Input: part model. Units: mm. Frame: model coordinates. A direction names the side the tool comes from. Coordinates: 2 decimals unless noted, no trailing zeros. Order: outer loops, then holes, each group sorted by start corner. A loop starts at its lowest first (then second) coordinate and runs counter-clockwise, first axis right, second up.
from build123d import *

# Parameters (mm, degrees)
SWEEP1_PROFILE_R = 9.5
CHAMFER1_SIZE    = 2


with BuildPart() as part:
    # Sweep1: sweep along a curve in space
    with BuildLine() as sweep1_path:
        Line((0, 0, 0), (0, 0, 40.5))
        ThreePointArc((0, 0, 40.5), (0, -11.569282143, 68.430717857), (0, -39.5, 80))
        Line((0, -39.5, 80), (0, -129.5, 80))
        ThreePointArc((0, -129.5, 80), (-11.569282143, -157.430717857, 80), (-39.5, -169, 80))
        Line((-39.5, -169, 80), (-84.5, -169, 80))
    # Sweep1 profile (on start of the path) → Sweep1 (sweep)
    with BuildSketch(Plane.XY):
        Circle(SWEEP1_PROFILE_R)
    sweep(path=sweep1_path.line)

    # Chamfer1
    chamfer1_edges = [part.edges().sort_by_distance(p)[0] for p in [
        (-84.5, -159.5, 80),
    ]]
    chamfer(chamfer1_edges, length=CHAMFER1_SIZE)


solid = part.part
Item 1: Cut plane A-A on z = 33. Return loops of the section in (x, y), then the cut area to 3 significant figures.
Response values:
outline: circle Ø19 at (0, 0)
area: 284 mm2
Item 2: Access query for faces 1 (the face through (-61.3, -174.11, 88.01)), 2 (the face through (-84.5, -169, 80)). Directions: +Z, -Z, +X, -X, +Y, -Y. A direction counts if a zero-diameter tool reaches every point of the face in a straight line with its end or side. Return the directions, or none.
Response values:
face 1: -X
face 2: +Z, -Z, -X, +Y, -Y
Item 3: Draft query along Y for faces 3 (the face through (0, 0, 0)), 4 (the face through (4.38, -8.43, 20.53)), 5 (the face through (-1.24, -85.13, 89.42)). Return one class per face: pulls with the +Y half, pulls with the -Y half, needs draft (parallel to the pull), parting line crosses it, or undercut.
Response values:
face 3: needs draft
face 4: parting line crosses it
face 5: undercut
Item 4: Ray query, probe 1 along X at (y, z) = (-114.5, 80); probe 2 along Z at (x, y) = (-5.5, -159.5); probe 3 along Z at (x, y) = (-5, -96). Return the intervals inside material, ascending.
Response values:
probe 1: x = -9.5 to 9.5
probe 2: z = 72.51 to 87.49
probe 3: z = 71.92 to 88.08
Item 5: Pin query (flat end, axial travel): pin 1 Ø10 at (y, z) = (-42.5, 72.5) entering from -X; pin 2 Ø2 at (x, y) = (-1.5, -80.5) entering from +Z. Return the tip coordinate at first contact, or that it passes through.
Response values:
pin 1: stops at x = -9.17
pin 2: stops at z = 89.49
Item 6: Cut plane B-B on x = -57.5. Return loops of the section in (y, z).
Response values:
outline: circle Ø19 at (-169, 80)
